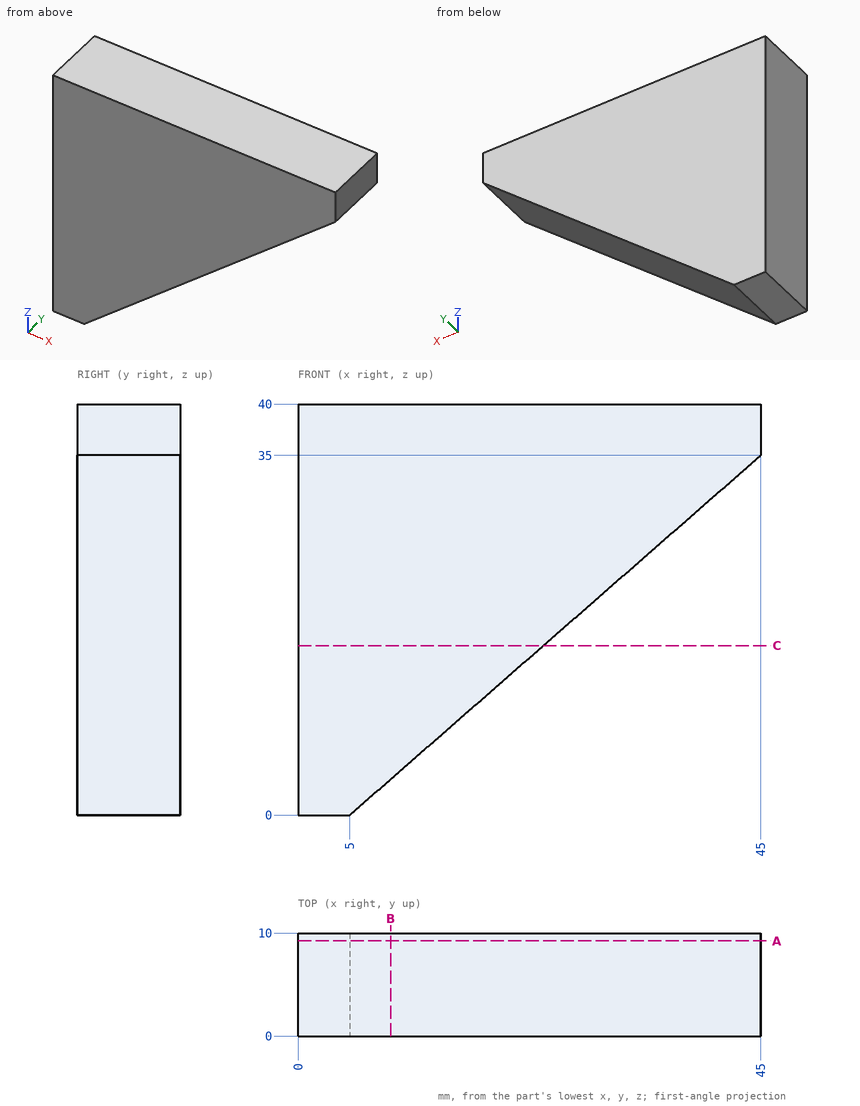
Design review of the part shown in the three views and the two pictorial views. Dimensions are in mm from the part's minimum x, y and z. Round coordinates to 2 decimals unless told otherwise and drop trailing zeros. Loops run counter-clockwise (first coordinate to the right, second up) from the corner with the lowest first, then second, coordinate; pieces in that order, holes last. Notation, with made-up numbers: M 46,15 L 65,15 A33 ccw 65,46 Z; hole C 66.25,75.25 d1. An arc over 180 degrees is marked long. Answer as a JSON object with one key per item and string values.
Item 1: We need section A-A on y = 9.25. Give the boundary of the cut face in (x, z).
Answer sheet:
{"outline": "M 0,0 L 5,0 L 45,35 L 45,40 L 0,40 Z"}
Item 2: We need section C-C on z = 16.5. Give the boundary of the cut face in (x, y), and give its area (3 significant figures).
Answer sheet:
{"outline": "M 0,0 L 23.86,0 L 23.86,10 L 0,10 Z", "area": "239 mm^2"}
Item 3: We need section B-B on x = 9. Give the boundary of the cut face in (y, z), and give its area (3 significant figures).
Answer sheet:
{"outline": "M 0,3.5 L 10,3.5 L 10,40 L 0,40 Z", "area": "365 mm^2"}
Item 4: Wall thickness on L1, parallel to Z at x = 42.5, y = 6.25; L2, parallel to Z at x = 14, y = 6 (3 decimals); L3, parallel to X at y = 7.25, z = 8.5: over which ranges is each line inside the solid? List them lowest first. Write a range as from..to.
Answer sheet:
{"L1": "z = 32.81..40", "L2": "z = 7.875..40", "L3": "x = 0..14.71"}
Item 5: Clearance check with flat-ended pins moving along their axes: P1, Ø2, axis at y = 8, z = 18.5, coming from the +X side; P2, Ø1.5, axis at y = 3, z = 6, coming from the +X side. State where each tip first meets the part, or that it passes through.
Answer sheet:
{"P1": "stops at x = 27.29", "P2": "stops at x = 12.71"}
